```python
from build123d import *

# Parameters (mm, degrees)
SKETCH_1_W             = 226
SKETCH_1_H             = 30
EXTRUDE_1_DEPTH        = 15
SKETCH_2_W             = 203
SKETCH_2_H             = 30
CUT_EXTRUDE_1_DEPTH    = 10
SKETCH_3_W             = 203
SKETCH_3_H             = 10
CUT_EXTRUDE_2_DEPTH    = 115.429017299
CUT_EXTRUDE_3_DEPTH    = 115.973910084
CUT_EXTRUDE_4_DEPTH    = 6
HOLE_WIZARD_M4_1_D     = 3.3
PATTERN_LINEAR_1_COUNT = 12
PATTERN_LINEAR_1_PITCH = 15
CHAMFER_1_SIZE         = 2
FILLET_1_R             = 3


with BuildPart() as part:
    # 草图1 → 凸台-拉伸1 (new body)
    with BuildSketch(Plane.XY):
        Rectangle(SKETCH_1_W, SKETCH_1_H)
    extrude(amount=EXTRUDE_1_DEPTH)

    # 草图2 → 切除-拉伸1 (cut)
    with BuildSketch(Plane.XY.offset(15)):
        Rectangle(SKETCH_2_W, SKETCH_2_H)
    extrude(amount=-CUT_EXTRUDE_1_DEPTH, mode=Mode.SUBTRACT)

    # 草图3 → 切除-拉伸2 (cut, through all)
    with BuildSketch(Plane.XY.offset(5)):
        with Locations((0, 10)):
            Rectangle(SKETCH_3_W, SKETCH_3_H)
    extrude(amount=-CUT_EXTRUDE_2_DEPTH, mode=Mode.SUBTRACT)

    # 草图4 → 切除-拉伸3 (cut, through all)
    with BuildSketch(Plane(origin=(0, 0, 0), x_dir=(-1, 0, 0), z_dir=(0, 0, -1))):
        with BuildLine():
            Line((104.75, -7.5), (104.75, 7.5))
            ThreePointArc((104.75, 7.5), (107.5, 10.25), (110.25, 7.5))
            Line((110.25, 7.5), (110.25, -7.5))
            ThreePointArc((110.25, -7.5), (107.5, -10.25), (104.75, -7.5))
        make_face()
        with BuildLine():
            Line((-110.25, -7.5), (-110.25, 7.5))
            ThreePointArc((-110.25, 7.5), (-107.5, 10.25), (-104.75, 7.5))
            Line((-104.75, 7.5), (-104.75, -7.5))
            ThreePointArc((-104.75, -7.5), (-107.5, -10.25), (-110.25, -7.5))
        make_face()
    extrude(amount=-CUT_EXTRUDE_3_DEPTH, mode=Mode.SUBTRACT)

    # 草图5 → 切除-拉伸4 (cut)
    with BuildSketch(Plane(origin=(0, 0, 0), x_dir=(-1, 0, 0), z_dir=(0, 0, -1))):
        with BuildLine():
            Line((102.5, -7.5), (102.5, 7.5))
            ThreePointArc((102.5, 7.5), (107.5, 12.5), (112.5, 7.5))
            Line((112.5, 7.5), (112.5, -7.5))
            ThreePointArc((112.5, -7.5), (107.5, -12.5), (102.5, -7.5))
        make_face()
        with BuildLine():
            Line((-112.5, -7.5), (-112.5, 7.5))
            ThreePointArc((-112.5, 7.5), (-107.5, 12.5), (-102.5, 7.5))
            Line((-102.5, 7.5), (-102.5, -7.5))
            ThreePointArc((-102.5, -7.5), (-107.5, -12.5), (-112.5, -7.5))
        make_face()
    extrude(amount=-CUT_EXTRUDE_4_DEPTH, mode=Mode.SUBTRACT)

    # M4 螺纹孔1 (through all)
    with Locations(Plane(origin=(0, 0, 0), x_dir=(-1, 0, 0), z_dir=(0, 0, -1))):
        with Locations((-81.5, -8)):
            hole_wizard_m4_1 = Hole(HOLE_WIZARD_M4_1_D / 2)

    # 阵列(线性)1: M4 螺纹孔1 ×12
    with Locations(*[(-i * PATTERN_LINEAR_1_PITCH, 0, 0) for i in range(1, PATTERN_LINEAR_1_COUNT)]):
        add(hole_wizard_m4_1, mode=Mode.SUBTRACT)

    # 倒角1
    chamfer_1_edges = [part.edges().sort_by_distance(p)[0] for p in [
        (101.5, 15, 7.5),
        (101.5, -15, 10),
        (-101.5, -15, 10),
        (-101.5, 15, 7.5),
        (113, -15, 7.5),
        (-113, -15, 7.5),
        (-113, 15, 7.5),
        (113, 15, 7.5),
    ]]
    chamfer(chamfer_1_edges, length=CHAMFER_1_SIZE)

    # 圆角1
    fillet_1_edges = [part.edges().sort_by_distance(p)[0] for p in [
        (-101.5, 5, 2.5),
        (101.5, 5, 2.5),
    ]]
    fillet(fillet_1_edges, radius=FILLET_1_R)


solid = part.part
```
Input: part model. Units: mm. Frame: model coordinates. A direction names the side the tool comes from. Round coordinates to 2 decimals unless told otherwise and drop trailing zeros. Loops run counter-clockwise (first coordinate to the right, second up) from the corner with the lowest first, then second, coordinate; pieces in that order, holes last. Notation, with made-up numbers: M 35,5.25 L 54,5.25 A5 ccw 54,11.25 Z; hole C -15,29.25 d1. An arc over 180 degrees is marked long. Answer in a Markdown table with one row per item. Add a question column.
1. Section B-B (x = 107.5). Output: boundary loops of the cut face in (y, z), and give its area (4 significant figures).
2. Ray query, probe 1 along X at (y, z) = (-4.5, 13); probe 2 along X at (y, z) = (4.5, 5.25); probe 3 along X at (y, z) = (12, 10). Return the intervals inside material, ascending.
3. Contact query for a flat-ended pin moving along its axis: pin 1 (11.5 mm diameter, centred on x = -1.5, y = -7, fed in from +Z). Output: stop coordinate, or through.
4. Section A-A (z = 8.25). Output: boundary loops of the cut face in (x, y).
5. Section D-D (x = 28). Output: boundary loops of the cut face in (y, z).
6. Mould query, pull axis Y, two halves, no side actions, for faces 4 (the face through (-107.44, 10.25, 10.44)), 5 (the face through (-107, 15, 7)), 6 (the face through (-1, -15, 4)), 7 (the face through (-101.5, 0, 9)). Classes: released by +Y, released by -Y, zero draft, split by the parting line, or undercut.
7. Set-up query: faces 1 (the face through (107, 15, 7)), 2 (the face through (112.5, 0, 3)), 3 (the face through (110.25, 0, 10)). Return all of +Z, -Z, +X, -X, +Y, -Y with unobstructed straight access to the full face (end or side cutting, diameter ignored); none if empty.
8. Section C-C (y = 1). Output: boundary loops of the cut face in (x, z), and give its area (3 significant figures).
Values follow:
| question | item | result |
|---|---|---|
| 1 | outline | M -15,0 L -12.5,0 L -12.5,6 L -10.25,6 L -10.25,15 L -15,15 Z; M 10.25,6 L 12.5,6 L 12.5,0 L 15,0 L 15,15 L 10.25,15 Z |
| 1 | area | 115.5 mm^2 |
| 2 | probe 1 | -113 to -110.25, -104.75 to -101.5, 101.5 to 104.75, 110.25 to 113 |
| 2 | probe 2 | -113 to -112.5, -102.5 to -101.5, 101.5 to 102.5, 112.5 to 113 |
| 2 | probe 3 | -113 to -101.5, 101.5 to 113 |
| 3 | pin 1 | z = 5 |
| 4 | outline | M -113,-13 L -111,-15 L -103.5,-15 L -101.5,-13 L -101.5,13 L -103.5,15 L -111,15 L -113,13 Z; M 101.5,-13 L 103.5,-15 L 111,-15 L 113,-13 L 113,13 L 111,15 L 103.5,15 L 101.5,13 Z; hole M -110.25,-7.5 A2.75 ccw -104.75,-7.5 L -104.75,7.5 A2.75 ccw -110.25,7.5 Z; hole M 104.75,-7.5 A2.75 ccw 110.25,-7.5 L 110.25,7.5 A2.75 ccw 104.75,7.5 Z |
| 5 | outline | M -15,0 L 5,0 L 5,5 L -15,5 Z |
| 6 | face 4 | undercut |
| 6 | face 5 | released by +Y |
| 6 | face 6 | released by -Y |
| 6 | face 7 | zero draft |
| 7 | face 1 | +Z, -Z, +X, -X, +Y |
| 7 | face 2 | -Z |
| 7 | face 3 | +Z, -Z |
| 8 | outline | M -113,0 L -112.5,0 L -112.5,6 L -110.25,6 L -110.25,15 L -113,15 Z; M -104.75,6 L -102.5,6 L -102.5,0 L 102.5,0 L 102.5,6 L 104.75,6 L 104.75,15 L 101.5,15 L 101.5,5 L -101.5,5 L -101.5,15 L -104.75,15 Z; M 110.25,6 L 112.5,6 L 112.5,0 L 113,0 L 113,15 L 110.25,15 Z |
| 8 | area | 1,140 mm^2 |
